```python
from build123d import *

# Parameters (mm, degrees)
SKETCH1_R           = 29
SKETCH1_R_2         = 20
BOSS_EXTRUDE1_DEPTH = 23
CHAMFER1_SIZE       = 2
SKETCH2_W           = 6
SKETCH2_H           = 12.436847424
CUT_EXTRUDE1_DEPTH  = 48.021271782
CIRPATTERN1_COUNT   = 4


with BuildPart() as part:
    # Sketch1 → Boss-Extrude1 (new body)
    with BuildSketch(Plane(origin=(0, 0, 0), x_dir=(1, 0, 0), z_dir=(0, 1, 0))):
        with Locations(Location((0, 0, 0), (0, 0, 270))):
            Circle(SKETCH1_R)
        with Locations(Location((0, 0, 0), (0, 0, 270))):
            Circle(SKETCH1_R_2, mode=Mode.SUBTRACT)
    extrude(amount=BOSS_EXTRUDE1_DEPTH)

    # Chamfer1
    chamfer1_edges = [part.edges().sort_by_distance(p)[0] for p in [
        (0, 0, -29),
        (0, 23, -29),
    ]]
    chamfer(chamfer1_edges, length=CHAMFER1_SIZE)

    # Sketch2 → Cut-Extrude1 (cut, through all)
    with BuildSketch(Plane(origin=(0, 23, 0), x_dir=(1, 0, 0), z_dir=(0, 1, 0))):
        with Locations((0, 32.218423712)):
            Rectangle(SKETCH2_W, SKETCH2_H)
    cut_extrude1 = extrude(amount=-CUT_EXTRUDE1_DEPTH, mode=Mode.SUBTRACT)

    # CirPattern1: Cut-Extrude1 ×4 about axis
    cirpattern1_axis = Axis((0, 0, 0), (0, 1, 0))
    for i in range(1, CIRPATTERN1_COUNT):
        add(cut_extrude1.rotate(cirpattern1_axis, i * 360 / CIRPATTERN1_COUNT), mode=Mode.SUBTRACT)


solid = part.part
```
Geometry: final body of the model. Coordinates: model frame, mm. A direction names the side the tool comes from. Coordinates: 2 decimals unless noted, no trailing zeros. Loops run counter-clockwise (first coordinate to the right, second up) from the corner with the lowest first, then second, coordinate; pieces in that order, holes last. Notation, with made-up numbers: (48.5, 66.25) -> (72.5, 66.25) arc R30 ccw to (72.5, 98.25) -> close; hole circle Ø11 at (-23, 78). An arc over 180 degrees is marked (long way). Use a Markdown table: item, result. Add a question column.
(1) Access query for faces 1 (the flat face through (27, 12, -3)), 2 (the flat face through (0, 12, 26)), 3 (the flat face through (-26, 12, 0)). Directions: +Z, -Z, +X, -X, +Y, -Y. A direction counts if a zero-diameter tool reaches every point of the face in a straight line with its end or side. Return the directions, or none.
(2) Section query B-B, the plane x = 0. Return loops of the section in (y, z), plus the area to 3 significant figures.
(3) Line query: line 1 along X through (y, z) = (5.25, 0); line 2 along X through (y, z) = (8, 2.5); line 3 along Z through (x, y) = (2, 9.25). Output: solid intervals per line, ascending.
(4) Pin query (flat end, axial travel): pin 1 Ø2 at (x, z) = (20, -0.5) entering from -Y; pin 2 Ø10 at (y, z) = (6.5, -14.5) entering from +X; pin 3 Ø1.4 at (y, z) = (10.5, 26.5) entering from +X; pin 4 Ø2.5 at (x, y) = (-27.5, 16) entering from -Z. Return the tip coordinate at first contact, or that it passes through.
(5) Section query C-C, the plane z = 0. Return loops of the section in (x, y), plus the area to 3 significant figures.
(6) Section query A-A, the plane y = 19. Return loops of the section in (x, z), plus the area to 3 significant figures.
(7) Mould query, pull axis X, two halves, no side actions, for faces 4 (the flat face through (0, 12, -26)), 5 (the flat face through (26, 12, 0)), 6 (the conical face through (-19.501, 22.681, 19.132)). Classes: pulls with the +X half, pulls with the -X half, needs draft (parallel to the pull), parting line crosses it, or undercut.
Answer:
| question | item | result |
|---|---|---|
| 1 | face 1 | +X, +Y, -Y |
| 1 | face 2 | +Z, +Y, -Y |
| 1 | face 3 | -X, +Y, -Y |
| 2 | outline | (0, -26) -> (23, -26) -> (23, -20) -> (0, -20) -> close; (0, 20) -> (23, 20) -> (23, 26) -> (0, 26) -> close |
| 2 | area | 276 mm^2 |
| 3 | line 1 | x = -26 to -20, 20 to 26 |
| 3 | line 2 | x = -26 to -19.84, 19.84 to 26 |
| 3 | line 3 | z = -26 to -19.9, 19.9 to 26 |
| 4 | pin 1 | stops at y = 0 |
| 4 | pin 2 | stops at x = 27.4 |
| 4 | pin 3 | stops at x = 13.24 |
| 4 | pin 4 | stops at z = -12.33 |
| 5 | outline | (-26, 0) -> (-20, 0) -> (-20, 23) -> (-26, 23) -> close; (20, 0) -> (26, 0) -> (26, 23) -> (20, 23) -> close |
| 5 | area | 276 mm^2 |
| 6 | outline | (-28.84, -3) arc R29 ccw to (-3, -28.84) -> (-3, -26) -> (3, -26) -> (3, -28.84) arc R29 ccw to (28.84, -3) -> (26, -3) -> (26, 3) -> (28.84, 3) arc R29 ccw to (3, 28.84) -> (3, 26) -> (-3, 26) -> (-3, 28.84) arc R29 ccw to (-28.84, 3) -> (-26, 3) -> (-26, -3) -> close; hole circle Ø40 at (0, 0) |
| 6 | area | 1,310 mm^2 |
| 7 | face 4 | undercut |
| 7 | face 5 | pulls with the +X half |
| 7 | face 6 | pulls with the -X half |
